Read the model definition and answer for the solid it produces. Units are mm, in the model's axes. Give positions to 0.01 mm unless a question says otherwise; leave off trailing zeros. Write each loop counter-clockwise with the first axis right and the second up, starting at its lowest first coordinate (ties: lowest second). Pieces come first, ordered by that corner, then holes. Notation, with made-up numbers: (-24, 64.25) -> (19, 64.25) arc R29 cw to (19, 101.25) -> close; hole circle Ø5 at (60, -22). An arc over 180 degrees is marked (long way). Use a Markdown table: item, result.
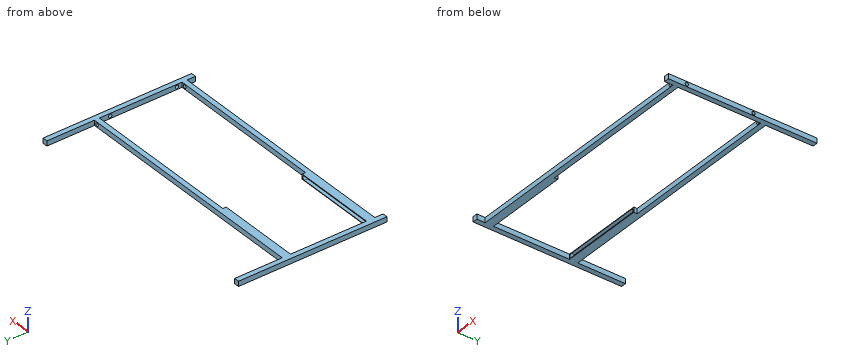
from build123d import *

# Parameters (mm, degrees)
SKETCH1_W             = 15
SKETCH1_H             = 15
BOSS_EXTRUDE1_DEPTH   = 445
BOSS_EXTRUDE1_2_DEPTH = 445
SKETCH2_W             = 15
SKETCH2_H             = 15
BOSS_EXTRUDE2_DEPTH   = 730
SKETCH3_R             = 5
CUT_EXTRUDE1_DEPTH    = 900
SKETCH4_W             = 250
SKETCH4_H             = 15
BOSS_EXTRUDE5_DEPTH   = 10
BOSS_EXTRUDE6_START   = 10
SKETCH6_W             = 250
SKETCH6_H             = 15
BOSS_EXTRUDE6_DEPTH   = 10
SKETCH7_R             = 5
CUT_EXTRUDE2_DEPTH    = 500


with BuildPart() as part:
    # Sketch1 → Boss-Extrude1 (new body)
    with BuildSketch(Plane(origin=(0, 0, 0), x_dir=(1, 0, 0), z_dir=(0, 1, 0))):
        Rectangle(SKETCH1_W, SKETCH1_H)
    extrude(amount=-BOSS_EXTRUDE1_DEPTH)



with BuildPart() as body_2:
    # Sketch1 → Boss-Extrude1 2 (new body)
    with BuildSketch(Plane(origin=(0, 0, 0), x_dir=(1, 0, 0), z_dir=(0, 1, 0))):
        with Locations((745, 0)):
            Rectangle(SKETCH1_W, SKETCH1_H)
    extrude(amount=-BOSS_EXTRUDE1_2_DEPTH)


with BuildPart() as part_1:
    add(part.part)

    add(body_2.part)  # Boss-Extrude2 merges body 2
    # Sketch2 → Boss-Extrude2 (add)
    with BuildSketch(Plane(origin=(7.5, 0, 0), x_dir=(0, 0, -1), z_dir=(1, 0, 0))):
        with Locations((0, -412.5)):
            Rectangle(SKETCH2_W, SKETCH2_H)
        with Locations((0, -150)):
            Rectangle(SKETCH2_W, SKETCH2_H)
    extrude(amount=BOSS_EXTRUDE2_DEPTH)

    # Sketch3 → Cut-Extrude1 (cut)
    with BuildSketch(Plane(origin=(7.5, 0, 0), x_dir=(0, 0, -1), z_dir=(1, 0, 0))):
        with Locations(Location((0, -190, 0), (0, 0, 180))):
            Circle(SKETCH3_R)
        with Locations(Location((0, -390, 0), (0, 0, 180))):
            Circle(SKETCH3_R)
    extrude(amount=CUT_EXTRUDE1_DEPTH, mode=Mode.SUBTRACT)

    # Sketch4 → Boss-Extrude5 (add)
    with BuildSketch(Plane(origin=(0, -405, 0), x_dir=(1, 0, 0), z_dir=(0, 1, 0))):
        with Locations((132.5, 0)):
            Rectangle(SKETCH4_W, SKETCH4_H)
        with BuildLine():
            ThreePointArc((15.7, -6), (9.7, 0), (15.7, 6))
            Line((15.7, 6), (249.3, 6))
            ThreePointArc((249.3, 6), (255.3, 0), (249.3, -6))
            Line((249.3, -6), (15.7, -6))
        make_face(mode=Mode.SUBTRACT)
    extrude(amount=BOSS_EXTRUDE5_DEPTH)

    # Sketch6 → Boss-Extrude6 (add)
    with BuildSketch(Plane.XZ.offset(157.5).offset(BOSS_EXTRUDE6_START)):
        with Locations((132.5, 0)):
            Rectangle(SKETCH6_W, SKETCH6_H)
        with BuildLine():
            ThreePointArc((15.7, -6), (9.7, 0), (15.7, 6))
            Line((15.7, 6), (249.3, 6))
            ThreePointArc((249.3, 6), (255.3, 0), (249.3, -6))
            Line((249.3, -6), (15.7, -6))
        make_face(mode=Mode.SUBTRACT)
    extrude(amount=-BOSS_EXTRUDE6_DEPTH)

    # Sketch7 → Cut-Extrude2 (cut)
    with BuildSketch(Plane(origin=(0, -142.5, 0), x_dir=(1, 0, 0), z_dir=(0, 1, 0))):
        with Locations(Location((727.5, 0, 0), (0, 0, 270))):
            Circle(SKETCH7_R)
    extrude(amount=-CUT_EXTRUDE2_DEPTH, mode=Mode.SUBTRACT)


solid = part_1.part
Item 1: A cutting plane is placed at C-C (z = 0). Count the separate pieces of the cut face and the enclosed holes in it, then the cut area to 3 significant figures.
Return value:
| item | result |
|---|---|
| separate pieces | 4 |
| enclosed holes | 0 |
| area | 34,700 mm^2 |
Item 2: Each of these flat-tipped pins is pushed along its axis until it touches: P1, Ø8, axis at x = 76, z = 2, coming from the +Y side; P2, Ø4.5, axis at x = 462, z = 3.5, coming from the -Y side. Where does it stop, or does it pass through?
Return value:
| item | result |
|---|---|
| P1 | y = -142.5 |
| P2 | y = -420 |
Item 3: A cutting plane is placed at D-D (x = 640.5). Give the vertices of the cut face in (y, z), then the cut area to 3 significant figures.
Return value:
| item | result |
|---|---|
| outline | (-420, -7.5) -> (-405, -7.5) -> (-405, 7.5) -> (-420, 7.5) -> close; (-157.5, -7.5) -> (-142.5, -7.5) -> (-142.5, 7.5) -> (-157.5, 7.5) -> close |
| area | 450 mm^2 |
Item 4: A cutting plane is placed at A-A (x = 130). Give the vertices of the cut face in (y, z).
Return value:
| item | result |
|---|---|
| outline | (-420, -7.5) -> (-395, -7.5) -> (-395, -6) -> (-405, -6) -> (-405, 6) -> (-395, 6) -> (-395, 7.5) -> (-420, 7.5) -> close; (-167.5, -7.5) -> (-142.5, -7.5) -> (-142.5, 7.5) -> (-167.5, 7.5) -> (-167.5, 6) -> (-157.5, 6) -> (-157.5, -6) -> (-167.5, -6) -> close |
Item 5: Straight lines are drawn through the part: line 1 along X through (y, z) = (-295, 1.25); line 2 along Y through (x, z) = (110.5, 1.25); line 3 along Y through (x, z) = (745, 0). For each, find the intervals that lie inside material, in ascending order. Write a range as [from, to].
Return value:
| item | result |
|---|---|
| line 1 | [-7.5, 7.5], [737.5, 752.5] |
| line 2 | [-420, -405], [-157.5, -142.5] |
| line 3 | [-445, -395], [-385, -195], [-185, 0] |
Item 6: A cutting plane is placed at B-B (y = -280.5). Give the vertices of the cut face in (x, z), then the cut area to 3 significant figures.
Return value:
| item | result |
|---|---|
| outline | (-7.5, -7.5) -> (7.5, -7.5) -> (7.5, 7.5) -> (-7.5, 7.5) -> close; (737.5, -7.5) -> (752.5, -7.5) -> (752.5, 7.5) -> (737.5, 7.5) -> close |
| area | 450 mm^2 |
